```python
from build123d import *

# Parameters (mm, degrees)
BASE_PLATE_SKETCH_W       = 200
BASE_PLATE_SKETCH_H       = 100
BASE_PLATE_DEPTH          = 10
RAISED_PAD_SKETCH_W       = 120
RAISED_PAD_SKETCH_H       = 100
RAISED_PAD_DEPTH          = 10
CORNER_CHAMFER_A_SIZE     = 20
CORNER_CHAMFER_B_SIZE     = 20
ADJUSTMENT_SLOTS_2X_DEPTH = 20
LUG_SKETCH_R              = 10
PIERCED_LUG_DEPTH         = 20
MOUNTING_HOLES_SKETCH_R   = 6
MOUNTING_HOLES_4X_DEPTH   = 20


with BuildPart() as part:
    # Base Plate Sketch → Base Plate (new body)
    with BuildSketch(Plane(origin=(0, 0, 0), x_dir=(1, 0, 0), z_dir=(0, 1, 0))):
        Rectangle(BASE_PLATE_SKETCH_W, BASE_PLATE_SKETCH_H)
    extrude(amount=BASE_PLATE_DEPTH)

    # Raised Pad Sketch → Raised Pad (add)
    with BuildSketch(Plane(origin=(0, 10, 0), x_dir=(1, 0, 0), z_dir=(0, 1, 0))):
        with Locations((-40, 0)):
            Rectangle(RAISED_PAD_SKETCH_W, RAISED_PAD_SKETCH_H)
    extrude(amount=RAISED_PAD_DEPTH)

    # Corner Chamfer A
    corner_chamfer_a_edges = [part.edges().sort_by_distance(p)[0] for p in [
        (100, 5, 50),
    ]]
    chamfer(corner_chamfer_a_edges, length=CORNER_CHAMFER_A_SIZE)

    # Corner Chamfer B
    corner_chamfer_b_edges = [part.edges().sort_by_distance(p)[0] for p in [
        (100, 5, -50),
    ]]
    chamfer(corner_chamfer_b_edges, length=CORNER_CHAMFER_B_SIZE)

    # Adjustment Slots Sketch → Adjustment Slots 2x (cut)
    with BuildSketch(Plane(origin=(0, 20, 0), x_dir=(1, 0, 0), z_dir=(0, 1, 0))):
        with BuildLine():
            Line((-50, -24), (0, -24))
            ThreePointArc((0, -24), (6, -30), (0, -36))
            Line((0, -36), (-50, -36))
            ThreePointArc((-50, -36), (-56, -30), (-50, -24))
        make_face()
        with BuildLine():
            Line((-50, 24), (0, 24))
            ThreePointArc((0, 24), (6, 30), (0, 36))
            Line((0, 36), (-50, 36))
            ThreePointArc((-50, 36), (-56, 30), (-50, 24))
        make_face()
    extrude(amount=-ADJUSTMENT_SLOTS_2X_DEPTH, mode=Mode.SUBTRACT)

    # Lug Sketch → Pierced Lug (add)
    with BuildSketch(Plane.ZY.offset(100)):
        with BuildLine():
            Line((-21.999787954, 71.874734943), (-50, 20))
            Line((-50, 20), (50, 20))
            Line((50, 20), (21.999787954, 71.874734943))
            ThreePointArc((21.999787954, 71.874734943), (0, 85), (-21.999787954, 71.874734943))
        make_face()
        with Locations((0, 60)):
            Circle(LUG_SKETCH_R, mode=Mode.SUBTRACT)
    extrude(amount=-PIERCED_LUG_DEPTH)

    # Mounting Holes Sketch → Mounting Holes 4x (cut)
    with BuildSketch(Plane(origin=(0, 10, 0), x_dir=(1, 0, 0), z_dir=(0, 1, 0))):
        with Locations(Location((40, 29.565570893, 0), (0, 0, 270))):
            Circle(MOUNTING_HOLES_SKETCH_R)
        with Locations(Location((80, 29.565570893, 0), (0, 0, 270))):
            Circle(MOUNTING_HOLES_SKETCH_R)
        with Locations(Location((80, -20.434429107, 0), (0, 0, 90))):
            Circle(MOUNTING_HOLES_SKETCH_R)
        with Locations(Location((40, -20.434429107, 0), (0, 0, 90))):
            Circle(MOUNTING_HOLES_SKETCH_R)
    extrude(amount=-MOUNTING_HOLES_4X_DEPTH, mode=Mode.SUBTRACT)


solid = part.part
```
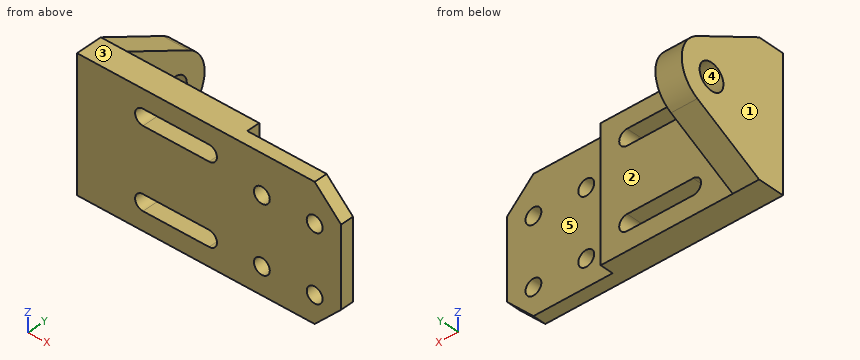
Geometry check sheet. Reference: the model listing, model coordinates, mm. Face numbers are marked on the shaded views. A direction names the side the tool comes from. Coordinates: 2 decimals unless noted, no trailing zeros. Loops run counter-clockwise (first coordinate to the right, second up) from the corner with the lowest first, then second, coordinate; pieces in that order, holes last.
Item 1: Go/stop test with flat-tipped pins: pin 1 Ø5 at (x, z) = (-57.5, -39) entering from +Y; pin 2 Ø6 at (x, z) = (-37.5, 9.5) entering from -Y; pin 3 Ø1 at (y, z) = (21, -31.5) entering from +X; pin 4 Ø19 at (x, z) = (40, -29.57) entering from +Y. Record where each tip stops, or that it passes through.
Item 2: Sectioned sample at D-D, the plane y = 60. Record the boundary of the cut face in (x, z).
Item 3: Release check for a two-part mould opening along Y. For the marked faces 3, 4 and 5 record: released by +Y, released by -Y, zero draft, split by the parting line, or undercut.
Item 4: Access from +Z, -Z, +X, -X, +Y, -Y to the whole of each face (thin tool, end or side, straight path). Record for the marked faces 1 and 2.
Item 5: Thickness scan on line 1 (X direction, y = 5.5, z = -31); line 2 (Y direction, x = -16, z = 3.5); line 3 (X direction, y = 52, z = -27). Record the ranges inside material, lowest first.
Item 6: Sectioned sample at C-C, the plane y = 8. Record the boundary of the cut face in (x, z).
Item 7: Sectioned sample at B-B, the plane z = 0. Record the boundary of the cut face in (x, y).
Item 8: Sectioned sample at A-A, the plane x = 40. Record the boundary of the cut face in (y, z), then the cut area to 3 significant figures.
Check result:
1. pin 1: stops at y = 20
1. pin 2: stops at y = 0
1. pin 3: stops at x = -80
1. pin 4: stops at y = 10
2. outline: (-100, -28.41) - (-80, -28.41) - (-80, -10) - (-100, -10) - close; (-100, 10) - (-80, 10) - (-80, 28.41) - (-100, 28.41) - close
3. face 3: zero draft
3. face 4: undercut
3. face 5: released by +Y
4. face 1: +Z, -Z, -X, +Y, -Y
4. face 2: +Z, -Z, +X, +Y
5. line 1: x = -100 to -55.92, 5.92 to 34.17, 45.83 to 74.17, 85.83 to 99
5. line 2: y = 0 to 20
5. line 3: x = -100 to -80
6. outline: (-100, -50) - (80, -50) - (100, -30) - (100, 30) - (80, 50) - (-100, 50) - close; hole (-50, -36) - (0, -36) arc R6 ccw to (0, -24) - (-50, -24) arc R6 ccw to start; hole (-50, 24) - (0, 24) arc R6 ccw to (0, 36) - (-50, 36) arc R6 ccw to start; hole circle Ø12 at (40, -29.57); hole circle Ø12 at (40, 20.43); hole circle Ø12 at (80, -29.57); hole circle Ø12 at (80, 20.43)
7. outline: (-100, 0) - (100, 0) - (100, 10) - (20, 10) - (20, 20) - (-80, 20) - (-80, 50) - (-100, 50) - close; (-100, 70) - (-80, 70) - (-80, 85) - (-100, 85) - close
8. outline: (0, -50) - (10, -50) - (10, -35.57) - (0, -35.57) - close; (0, -23.57) - (10, -23.57) - (10, 14.43) - (0, 14.43) - close; (0, 26.43) - (10, 26.43) - (10, 50) - (0, 50) - close
8. area: 760 mm2
